from build123d import *

# Parameters (mm, degrees)
BIG_END_EYE_SKETCH_R        = 20
BIG_END_EYE_SKETCH_R_2      = 15
BIG_END_EYE_40_DEPTH        = 7
SMALL_END_EYE_SKETCH_R      = 9.25
SMALL_END_EYE_SKETCH_R_2    = 7.625
SMALL_END_EYE_18_5_DEPTH    = 7
SHANK_DEPTH                 = 4
BIG_END_BLEND_R26_65_A_R    = 26.65
SMALL_END_BLEND_R15_25_A_R  = 15.25
SMALL_END_BLEND_R15_25_B_R  = 15.25
BIG_END_BLEND_R26_65_B_R    = 26.65
SHANK_RECESS_2_5_DEEP_DEPTH = 2.5
SHANK_PAD_2_5_DEPTH         = 2.5


with BuildPart() as part:
    # Big End Eye Sketch → Big End Eye Ø40 (new, symmetric)
    with BuildSketch(Plane(origin=(0, 0, 0), x_dir=(1, 0, 0), z_dir=(0, 1, 0))):
        with Locations(Location((47.5, 0, 0), (0, 0, 270))):
            Circle(BIG_END_EYE_SKETCH_R)
        with Locations(Location((47.5, 0, 0), (0, 0, 270))):
            Circle(BIG_END_EYE_SKETCH_R_2, mode=Mode.SUBTRACT)
    extrude(amount=BIG_END_EYE_40_DEPTH, both=True)



with BuildPart() as body_2:
    # Small End Eye Sketch → Small End Eye Ø18.5 (new, symmetric)
    with BuildSketch(Plane(origin=(0, 0, 0), x_dir=(1, 0, 0), z_dir=(0, 1, 0))):
        with Locations(Location((-47.5, 0, 0), (0, 0, 270))):
            Circle(SMALL_END_EYE_SKETCH_R)
        with Locations(Location((-47.5, 0, 0), (0, 0, 270))):
            Circle(SMALL_END_EYE_SKETCH_R_2, mode=Mode.SUBTRACT)
    extrude(amount=SMALL_END_EYE_18_5_DEPTH, both=True)


with BuildPart() as part_1:
    add(part.part)

    add(body_2.part)  # Shank merges body 2
    # Shank Profile Sketch → Shank (add, symmetric)
    with BuildSketch(Plane(origin=(0, 0, 0), x_dir=(1, 0, 0), z_dir=(0, 1, 0))):
        Polygon((27.282550476, 4), (28.047385708, 4), (28.047385708, -4), (-38.306518326, -4), (-39.375179325, -4), (-39.375179325, 4), align=None)
    extrude(amount=SHANK_DEPTH, both=True)

    # Big End Blend R26.65 A
    big_end_blend_r26_65_a_edges = [part_1.edges().sort_by_distance(p)[0] for p in [
        (27.904082058, 0, -4),
    ]]
    fillet(big_end_blend_r26_65_a_edges, radius=BIG_END_BLEND_R26_65_A_R)

    # Small End Blend R15.25 A
    small_end_blend_r15_25_a_edges = [part_1.edges().sort_by_distance(p)[0] for p in [
        (-39.159586341, 0, -4),
    ]]
    fillet(small_end_blend_r15_25_a_edges, radius=SMALL_END_BLEND_R15_25_A_R)

    # Small End Blend R15.25 B
    small_end_blend_r15_25_b_edges = [part_1.edges().sort_by_distance(p)[0] for p in [
        (-39.159586341, 0, 4),
    ]]
    fillet(small_end_blend_r15_25_b_edges, radius=SMALL_END_BLEND_R15_25_B_R)

    # Big End Blend R26.65 B
    big_end_blend_r26_65_b_edges = [part_1.edges().sort_by_distance(p)[0] for p in [
        (27.904082058, 0, 4),
    ]]
    fillet(big_end_blend_r26_65_b_edges, radius=BIG_END_BLEND_R26_65_B_R)

    # Shank Recess Sketch → Shank Recess 2.5 Deep (cut)
    with BuildSketch(Plane(origin=(0, 4, 0), x_dir=(1, 0, 0), z_dir=(0, 1, 0))):
        with BuildLine():
            ThreePointArc((-35.01, 2.277583754), (-37.287583754, 0), (-35.01, -2.277583754))
            Line((-35.01, -2.277583754), (-35.01, -2.318344298))
            Line((-35.01, -2.318344298), (16.571994255, -3.074327461))
            ThreePointArc((16.571994255, -3.074327461), (20.473294407, -0.381788318), (17.33, 3.16639575))
            Line((17.33, 3.16639575), (17.33, 3.190774264))
            Line((17.33, 3.190774264), (-35.01, 2.28421045))
            Line((-35.01, 2.28421045), (-35.01, 2.277583754))
        make_face()
    extrude(amount=-SHANK_RECESS_2_5_DEEP_DEPTH, mode=Mode.SUBTRACT)

    # Shank Pad Sketch → Shank Pad 2.5 (add)
    with BuildSketch(Plane(origin=(0, 7, 0), x_dir=(1, 0, 0), z_dir=(0, 1, 0))):
        with BuildLine():
            Line((-38.413384426, 0), (-36.90605517, 0))
            Line((-36.90605517, 0), (-35.79105517, 0))
            ThreePointArc((-35.79105517, 0), (-36.117631109, 0.788424061), (-36.90605517, 1.115))
            Line((-36.90605517, 1.115), (-38.413384426, 1.115))
            Line((-38.413384426, 1.115), (-38.413384426, 0))
        make_face()
        with BuildLine():
            Line((-35.79105517, 0), (-36.90605517, 0))
            Line((-36.90605517, 0), (-38.413384426, 0))
            Line((-38.413384426, 0), (-38.413384426, -1.115))
            Line((-38.413384426, -1.115), (-36.90605517, -1.115))
            ThreePointArc((-36.90605517, -1.115), (-36.117631109, -0.788424061), (-35.79105517, 0))
        make_face()
    extrude(amount=-SHANK_PAD_2_5_DEPTH)


solid = part_1.part
Here's how the part is built. I have some questions about the finished solid (model axes, mm). A direction names the side the tool comes from. Round coordinates to 2 decimals unless told otherwise and drop trailing zeros. Write each loop counter-clockwise with the first axis right and the second up, starting at its lowest first coordinate (ties: lowest second). Pieces come first, ordered by that corner, then holes.
1. For faces 1 (the cylindrical face through (23.223, 0.056, -6.327)), 2 (the cylindrical face through (23.513, 0.056, 6.459)), 3 (the cylindrical face through (20.463, 2.768, 0.456)), 4 (the cylindrical face through (62.372, -0.098, -1.953)), which set-ups out of +Z, -Z, +X, -X, +Y, -Y let a thin tool reach every point of the face, with its end or its side?
2. Will these pins go through, and if not, where does the flat tip stop? pin 1 Ø10 at (x, z) = (17.33, 0) entering from -Y; pin 2 Ø8 at (x, y) = (-32.5, 4) entering from +Z; pin 3 Ø5 at (x, y) = (8.5, 2.5) entering from -Z.
3. Suppose I cut it at B-B (z = -10.5). List the corners of the cut face in (x, y) for me, and give its area (3 significant figures).
4. I need wall thicknesses on L1, parallel to X at y = -2.5, z = 0 (3 decimals); L2, parallel to X at y = 2.85, z = 0 (3 decimals); L3, parallel to X at y = 5.25, z = -5. Which ranges of each line are inside material? Lowest first, please.
5. If we mould it in two halves opening along X, with no side actions, what happens to faces 5 (the cylindrical face through (-37.287, 2.768, -0.05)), 6 (the flat face through (-5, 4, -3)), 7 (the flat face through (62.4, -7, 2.9))? For each: released by +X, released by -X, zero draft, split by the parting line, or undercut.
6. Suppose I cut it at A-A (x = -47.5). List the corners of the cut face in (y, z) for me (3 decimals).
7. Suppose I cut it at C-C (x = 47.5). List the corners of the cut face in (y, z) for me, and give its area (3 significant figures).
8. Suppose I cut it at D-D (x = 6.5). List the corners of the cut face in (y, z) for me, and give its area (3 significant figures).
Answer sheet:
1. face 1: -Z, +Y, -Y
1. face 2: +Z, +Y, -Y
1. face 3: +Y
1. face 4: +Y, -Y
2. pin 1: stops at y = -4
2. pin 2: stops at z = 4.58
2. pin 3: stops at z = -4
3. outline: (29.77, -4) - (30.48, -4) - (30.48, -7) - (36.79, -7) - (36.79, 7) - (30.48, 7) - (30.48, 4) - (29.77, 4) - close; (58.21, -7) - (64.52, -7) - (64.52, 7) - (58.21, 7) - close
3. area: 182 mm2
4. L1: x = -56.75 to -55.125, -39.875 to 32.5, 62.5 to 67.5
4. L2: x = -56.75 to -55.125, -39.875 to -37.288, 20.496 to 32.5, 62.5 to 67.5
4. L3: x = -55.28 to -53.26, -41.74 to -39.72, 28.14 to 33.36, 61.64 to 66.86
5. face 5: undercut
5. face 6: undercut
5. face 7: zero draft
6. outline: (-7, -9.25) - (7, -9.25) - (7, -7.625) - (-7, -7.625) - close; (-7, 7.625) - (7, 7.625) - (7, 9.25) - (-7, 9.25) - close
7. outline: (-7, -20) - (7, -20) - (7, -15) - (-7, -15) - close; (-7, 15) - (7, 15) - (7, 20) - (-7, 20) - close
7. area: 140 mm2
8. outline: (-4, -4) - (4, -4) - (4, -3) - (1.5, -3) - (1.5, 2.93) - (4, 2.93) - (4, 4) - (-4, 4) - close
8. area: 49.2 mm2
